```python
from build123d import *

# Parameters (mm, degrees)
SKETCH1_W           = 90
SKETCH1_H           = 50
SKETCH1_R           = 5
BOSS_EXTRUDE1_DEPTH = 12
SKETCH2_R           = 15
BOSS_EXTRUDE2_DEPTH = 360


with BuildPart() as part:
    # Sketch1 → Boss-Extrude1 (new body)
    with BuildSketch(Plane.XY):
        Rectangle(SKETCH1_W, SKETCH1_H)
        with Locations((-30, 15)):
            Circle(SKETCH1_R, mode=Mode.SUBTRACT)
        with Locations((-30, -15)):
            Circle(SKETCH1_R, mode=Mode.SUBTRACT)
        with Locations((30, -15)):
            Circle(SKETCH1_R, mode=Mode.SUBTRACT)
        with Locations((30, 15)):
            Circle(SKETCH1_R, mode=Mode.SUBTRACT)
    extrude(amount=BOSS_EXTRUDE1_DEPTH)

    # Sketch2 → Boss-Extrude2 (add)
    with BuildSketch(Plane.XY.offset(12)):
        with Locations(Location((0, 0, 0), (0, 0, 180))):
            Circle(SKETCH2_R)
    extrude(amount=BOSS_EXTRUDE2_DEPTH)


solid = part.part
```
Check sheet for the modelled part. Datum: model origin and axes. Units: mm. A direction names the side the tool comes from. Coordinates: 2 decimals unless noted, no trailing zeros. Write each loop counter-clockwise with the first axis right and the second up, starting at its lowest first coordinate (ties: lowest second). Pieces come first, ordered by that corner, then holes. Notation, with made-up numbers: M 29.25,-31.5 L 60.25,-31.5 A27 ccw 60.25,5.5 Z; hole C 35.5,69 d8. An arc over 180 degrees is marked long. Write item = value, one per line. Start each with the question number.
1. Sectioned sample at B-B (y = 0). Record the cut outline in (x, z), then the cut area to 3 significant figures.
2. Go/stop test with flat-tipped pins: pin 1 (5 mm diameter, centred on x = 33.5, y = 10, fed in from +Z); pin 2 (5 mm diameter, centred on y = 3, z = 137.5, fed in from +X); pin 3 (5 mm diameter, centred on y = 10, z = 212.5, fed in from -X). Record where each tip stops, or that it passes through.
3. Thickness scan on probe 1 along Y at (x, z) = (-30, 8); probe 2 along Z at (x, y) = (-26, -21); probe 3 along X at (y, z) = (-1, 36). Record the ranges inside material, lowest first.
4. Mould release check, pull along X, two halves, no side actions. Record for faces 3 (the flat face through (-45, 0, 6)), 4 (the flat face through (-1, 0, 0)), 5 (the cylindrical face through (-34, 12, 6)): pulls with the +X half, pulls with the -X half, needs draft (parallel to the pull), parting line crosses it, or undercut.
5. Sectioned sample at C-C (x = 0). Record the cut outline in (y, z).
6. Sectioned sample at D-D (z = 58.5). Record the cut outline in (x, y), then the cut area to 3 significant figures.
7. Sectioned sample at A-A (x = 30). Record the cut outline in (y, z).
8. Tool access check on faces 1 (the cylindrical face through (26, 12, 6)), 2 (the cylindrical face through (-8.06, -12.65, 189.48)). Record the directions out of +Z, -Z, +X, -X, +Y, -Y that give a thin tool (end or side, any length) a straight path to the whole face; none if there is none.
The answers:
q1.outline = M -45,0 L 45,0 L 45,12 L 15,12 L 15,372 L -15,372 L -15,12 L -45,12 Z
q1.area = 11,900 mm²
q2.pin_1 = 12
q2.pin_2 = 14.99
q2.pin_3 = -12.99
q3.probe_1 = -25 to -20, -10 to 10, 20 to 25
q3.probe_2 = 0 to 12
q3.probe_3 = -14.97 to 14.97
q4.face_3 = pulls with the -X half
q4.face_4 = needs draft
q4.face_5 = undercut
q5.outline = M -25,0 L 25,0 L 25,12 L 15,12 L 15,372 L -15,372 L -15,12 L -25,12 Z
q6.outline = C 0,0 d30
q6.area = 707 mm²
q7.outline = M -25,0 L -20,0 L -20,12 L -25,12 Z; M -10,0 L 10,0 L 10,12 L -10,12 Z; M 20,0 L 25,0 L 25,12 L 20,12 Z
q8.face_1 = +Z, -Z
q8.face_2 = +Z
